Geometry: final body of the model. Coordinates: model frame, mm. A direction names the side the tool comes from. Give positions to 0.01 mm unless a question says otherwise; leave off trailing zeros. Loops run counter-clockwise (first coordinate to the right, second up) from the corner with the lowest first, then second, coordinate; pieces in that order, holes last. Notation, with made-up numbers: (81.5, 86) -> (116.5, 86) arc R25 cw to (116.5, 113) -> close; hole circle Ø2 at (68, -11.75). An arc over 180 degrees is marked (long way). One line per question, with ' | ' between items. Start each with the question number.
Item 1: Set-up query: faces 5 (the flat face through (-1, -22, 0)), 6 (the flat face through (16, -60, 17)), 7 (the flat face through (20, -65, -24)). Return all of +Z, -Z, +X, -X, +Y, -Y with unobstructed straight access to the full face (end or side cutting, diameter ignored); none if empty.
Item 2: Section A-A on z = 24. Return loops of the section in (x, y).
Item 3: Mould query, pull axis X, two halves, no side actions, for faces 1 (the flat face through (38, -65, -24)), 2 (the flat face through (-38, -65, -23)), 3 (the flat face through (-37, -84, 3)), 4 (the cylindrical face through (-58.541, -34.068, 17.745)). Classes: released by +X, released by -X, zero draft, split by the parting line, or undercut.
Item 4: Section C-C on y = -68. Give the number of separate pieces and of enclosed holes in the cut face, then the cut area to 3 significant figures.
Item 5: Section D-D on z = -2.5. Return loops of the section in (x, y).
Item 6: Material intervals for line 1 along X through (y, z) = (-52, 10.5); line 2 along Y through (x, z) = (-57.5, 27); line 3 along Y through (x, z) = (64, 11), sorted ascending. Write a range as [from, to].
Item 7: Section B-B on x = 61.5. Return loops of the section in (y, z).
Item 8: Pin query (flat end, axial travel): P1, Ø1.5, axis at x = 35.5, y = -58, coming from the -Z side; P2, Ø8, axis at x = 27, z = -7, coming from the +Y side; P3, Ø6, axis at x = -31, y = -61.5, coming from the -Z side. Return the tip coordinate at first contact, or that it passes through.
from build123d import *

# Parameters (mm, degrees)
BASE_BLOCK_DEPTH         = 35
BORE_PROFILE_R           = 20
BORE_40_DEPTH            = 35
MOUNTING_HOLES_PROFILE_R = 8
MOUNTING_HOLES_4X_DEPTH  = 35
SIDE_ARM_PROFILE_R       = 8
SIDE_ARM_DEPTH           = 18
LUG_START                = 18
LUG_BOSS_PROFILE_R       = 8
LUG_BOSS_DEPTH           = 18
RELIEF_CUT_PROFILE_W     = 32
RELIEF_CUT_PROFILE_H     = 48
RELIEF_CUT_DEPTH         = 35
BORE_CHAMFER_1MM_SIZE    = 1


with BuildPart() as part:
    # Base Block Profile → Base Block (new body)
    with BuildSketch(Plane.XY):
        with BuildLine():
            Line((-70, -28), (-70, -84))
            Line((-70, -84), (70, -84))
            Line((70, -84), (70, -28))
            ThreePointArc((70, -28), (47.647244828, -21.260291625), (38, 0))
            ThreePointArc((38, 0), (0, 38), (-38, 0))
            ThreePointArc((-38, 0), (-47.647244828, -21.260291625), (-70, -28))
        make_face()
    extrude(amount=BASE_BLOCK_DEPTH)

    # Bore Profile → Bore Ø40 (cut)
    with BuildSketch(Plane.XY.offset(35)):
        Circle(BORE_PROFILE_R)
    extrude(amount=-BORE_40_DEPTH, mode=Mode.SUBTRACT)

    # Mounting Holes Profile → Mounting Holes 4x (cut)
    with BuildSketch(Plane.XY.offset(35)):
        with Locations((-57.5, -42)):
            Circle(MOUNTING_HOLES_PROFILE_R)
        with Locations((-57.5, -70)):
            Circle(MOUNTING_HOLES_PROFILE_R)
        with Locations((57.5, -42)):
            Circle(MOUNTING_HOLES_PROFILE_R)
        with Locations((57.5, -70)):
            Circle(MOUNTING_HOLES_PROFILE_R)
    extrude(amount=-MOUNTING_HOLES_4X_DEPTH, mode=Mode.SUBTRACT)

    # Side Arm Profile → Side Arm (add)
    with BuildSketch(Plane(origin=(38, 0, 0), x_dir=(0, 0, -1), z_dir=(1, 0, 0))):
        with BuildLine():
            Line((0, -84), (0, -36))
            Line((0, -36), (50.096296037, -52.833333698))
            ThreePointArc((50.096296037, -52.833333698), (60.790292284, -70.581989463), (45, -84))
            Line((45, -84), (0, -84))
        make_face()
        with Locations((45, -68)):
            Circle(SIDE_ARM_PROFILE_R, mode=Mode.SUBTRACT)
    extrude(amount=-SIDE_ARM_DEPTH)

    # Lug Boss Profile → Lug Boss (add)
    with BuildSketch(Plane(origin=(-38, 0, 0), x_dir=(0, 0, -1), z_dir=(1, 0, 0)).offset(LUG_START)):
        with BuildLine():
            Line((0, -36), (0, -84))
            Line((0, -84), (45, -84))
            ThreePointArc((45, -84), (60.790292284, -70.581989463), (50.096296037, -52.833333698))
            Line((50.096296037, -52.833333698), (0, -36))
        make_face()
        with Locations((45, -68)):
            Circle(LUG_BOSS_PROFILE_R, mode=Mode.SUBTRACT)
    extrude(amount=-LUG_BOSS_DEPTH)

    # Relief Cut Profile → Relief Cut (cut)
    with BuildSketch(Plane(origin=(0, 0, 0), x_dir=(-1, 0, 0), z_dir=(0, 0, -1))):
        with Locations((0, -60)):
            Rectangle(RELIEF_CUT_PROFILE_W, RELIEF_CUT_PROFILE_H)
    extrude(amount=-RELIEF_CUT_DEPTH, mode=Mode.SUBTRACT)

    # Bore Chamfer 1mm
    bore_chamfer_1mm_edges = [part.edges().sort_by_distance(p)[0] for p in [
        (-20, 0, 0),
    ]]
    chamfer(bore_chamfer_1mm_edges, length=BORE_CHAMFER_1MM_SIZE)


solid = part.part
Result sheet:
1) face 5: -Z, +Y | face 6: +Z, -Z, -Y | face 7: -Z, +Y, -Y
2) outline: (-70, -84) -> (-16, -84) -> (-16, -36) -> (16, -36) -> (16, -84) -> (70, -84) -> (70, -28) arc R28.25 cw to (38, 0) arc R38 ccw to (-38, 0) arc R28.25 cw to (-70, -28) -> close; hole circle Ø16 at (-57.5, -70); hole circle Ø16 at (-57.5, -42); hole circle Ø40 at (0, 0); hole circle Ø16 at (57.5, -70); hole circle Ø16 at (57.5, -42)
3) face 1: released by +X | face 2: released by -X | face 3: zero draft | face 4: undercut
4) separate pieces: 6 | enclosed holes: 0 | area: 4,320 mm²
5) outline: (-38, -84) -> (-20, -84) -> (-20, -36.84) -> (-38, -36.84) -> close; (20, -84) -> (38, -84) -> (38, -36.84) -> (20, -36.84) -> close
6) line 1: x = [-70, -16], [16, 70] | line 2: y = [-84, -78], [-62, -50], [-34, -26.86] | line 3: y = [-84, -74.66], [-65.34, -46.66], [-37.34, -28.16]
7) outline: (-84, 0) -> (-76.93, 0) -> (-76.93, 35) -> (-84, 35) -> close; (-63.07, 0) -> (-48.93, 0) -> (-48.93, 35) -> (-63.07, 35) -> close; (-35.07, 0) -> (-27.85, 0) -> (-27.85, 35) -> (-35.07, 35) -> close
8) P1: stops at z = -58.06 | P2: stops at y = -37.01 | P3: stops at z = -60.61
